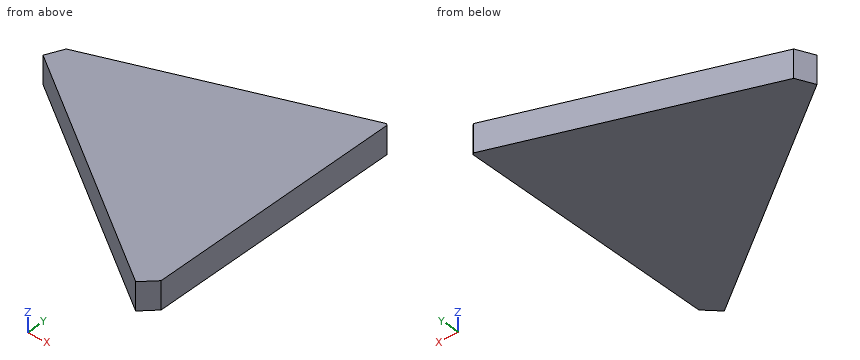
```python
from build123d import *
from OCP.BRepFilletAPI import BRepFilletAPI_MakeChamfer

# Parameters (mm, degrees)
EXTRUDE_START   = -260
EXTRUDE_1_DEPTH = 12
CHAMFER_1_SIZE  = 10
CHAMFER_1_SIZE2 = 7.180150431


with BuildPart() as part:
    # 草图1 → 凸台-拉伸1 (new body)
    with BuildSketch(Plane.XY.offset(EXTRUDE_START)):
        Polygon((-0.819152044, 243.432836403), (-115.534439314, 201.679886421), (0, 120.78180109), (0, 242.859259966), align=None)
    extrude(amount=EXTRUDE_1_DEPTH)

    # 倒角1: one chamfer whose edges measure the first distance from different faces: ONE call of the kernel's chamfer builder (chamfer() names one face for all edges)
    chamfer_1_edges_1 = [part.edges().sort_by_distance(p)[0] for p in [
        (0, 120.78180109, -254),
    ]]
    chamfer_1_side_1 = [part.faces().sort_by_distance(p)[0] for p in [
        (0, 181.820530528, -254),
    ]]
    chamfer_1_edges_2 = [part.edges().sort_by_distance(p)[0] for p in [
        (-115.534439314, 201.679886421, -254),
    ]]
    chamfer_1_side_2 = [part.faces().sort_by_distance(p)[0] for p in [
        (-58.176795679, 222.556361412, -254),
    ]]
    chamfer_1 = BRepFilletAPI_MakeChamfer(part.part.solid().wrapped)
    for e in chamfer_1_edges_1:
        chamfer_1.Add(CHAMFER_1_SIZE, CHAMFER_1_SIZE2, e.wrapped, chamfer_1_side_1[0].wrapped)  # the first distance lies on this face
    for e in chamfer_1_edges_2:
        chamfer_1.Add(CHAMFER_1_SIZE, CHAMFER_1_SIZE2, e.wrapped, chamfer_1_side_2[0].wrapped)  # the first distance lies on this face
    add(Compound.cast(chamfer_1.Shape()), mode=Mode.REPLACE)


solid = part.part
```
The model under review builds one solid part; all positions refer to its coordinate system, in mm. Round coordinates to 2 decimals unless told otherwise and drop trailing zeros. Loops run counter-clockwise (first coordinate to the right, second up) from the corner with the lowest first, then second, coordinate; pieces in that order, holes last. Notation, with made-up numbers: (-13, 22) -> (-9, 22) arc R20 ccw to (-9, 45) -> close; hole circle Ø4 at (41, 0.25). An arc over 180 degrees is marked (long way). Answer as a JSON object with one key per item and string values. Group by question number.
1) We need section C-C on y = 216. Write out the cut boundary in (x, z), then the cut area to 3 significant figures.
2) For line 1 (X direction, y = 193.5, z = -256.25); line 2 (X direction, y = 133, z = -250); line 3 (Y direction, x = -17.5, z = -256.25), list the stretches that pass through material, from the lowest coordinate up. Write a range as [from, to].
3) For pin 1 Ø5 at (x, z) = (-82.5, -257.5) entering from -Y; pin 2 Ø6 at (x, z) = (-68.5, -252.5) entering from -Y, all flat-tipped, find the tip position at first contact; note any pin that passes through.
4) We need section B-B on x = -98. Write out the cut boundary in (y, z).
5) We need section A-A on z = -254.75. Write out the cut boundary in (x, y), then the cut area to 3 significant figures.
Result set:
{
 "1": {"outline": "(-76.19, -260) -> (0, -260) -> (0, -248) -> (-76.19, -248) -> close", "area": "914 mm²"},
 "2": {"line 1": "[-103.85, 0]", "line 2": "[-17.45, 0]", "line 3": "[133.04, 237.36]"},
 "3": {"pin 1": "y = 176.8", "pin 2": "y = 166.65"},
 "4": {"outline": "(189.4, -260) -> (208.06, -260) -> (208.06, -248) -> (189.4, -248) -> close"},
 "5": {"outline": "(-109.65, 197.56) -> (-5.88, 124.9) -> (0, 130.78) -> (0, 242.86) -> (-0.82, 243.43) -> (-106.14, 205.1) -> close", "area": "7,040 mm²"}
}
